Input: part model. Units: mm. Frame: model coordinates. Face numbers are marked on the shaded views. A direction names the side the tool comes from. Give positions to 0.01 mm unless a question says otherwise; leave off trailing zeros. Write each loop counter-clockwise with the first axis right and the second up, starting at its lowest first coordinate (ties: lowest second). Pieces come first, ordered by that corner, then holes. Notation, with made-up numbers: (33.5, 71.5) -> (77.5, 71.5) arc R31 cw to (77.5, 100.5) -> close; hole circle Ø7 at (48, -38). An arc over 180 degrees is marked (long way). Return JSON: item names as keys, results as strings. Group by question number.
Item 1: Section B-B, the plane x = 0. Return loops of the section in (y, z).
Item 2: Line query: line 1 (Y direction, x = -1.1, z = -1.85); line 2 (X direction, y = 2, z = 1.15); line 3 (X direction, y = 2.25, z = 0.55). Output: solid intervals per line, ascending. Write a range as [from, to].
Item 3: Section C-C, the plane y = -0.25. Return loops of the section in (x, z).
Item 4: Mould query, pull axis X, two halves, no side actions, for the marked faces 4, 5 and 6. Classes: released by +X, released by -X, zero draft, split by the parting line, or undercut.
Item 5: Set-up query: the marked faces 1, 2 and 3. Return all of +Z, -Z, +X, -X, +Y, -Y with unobstructed straight access to the full face (end or side cutting, diameter ignored); none if empty.
Item 6: Section A-A, the plane y = 2. Return loops of the section in (x, z).
from build123d import *

# Parameters (mm, degrees)
SKETCH_1_R          = 2.75
EXTRUDE_1_DEPTH     = 3
CUT_EXTRUDE_1_DEPTH = 1.3
FILLET_1_R          = 0.15
SKETCH_5_R          = 1.5
EXTRUDE_2_DEPTH     = 8
CHAMFER_2_SIZE      = 0.28


with BuildPart() as part:
    # 草图1 → 凸台-拉伸1 (new body)
    with BuildSketch(Plane(origin=(0, 0, 0), x_dir=(1, 0, 0), z_dir=(0, 1, 0))):
        with Locations(Location((0, 0, 0), (0, 0, 270))):
            Circle(SKETCH_1_R)
    extrude(amount=EXTRUDE_1_DEPTH)

    # 草图2 → 切除-拉伸1 (cut)
    with BuildSketch(Plane(origin=(0, 3, 0), x_dir=(1, 0, 0), z_dir=(0, 1, 0))):
        Polygon((1.478016689, 0), (0.739008345, 1.28), (-0.739008345, 1.28), (-1.478016689, 0), (-0.739008345, -1.28), (0.739008345, -1.28), align=None)
    extrude(amount=-CUT_EXTRUDE_1_DEPTH, mode=Mode.SUBTRACT)

    # 圆角1
    fillet_1_edges = [part.edges().sort_by_distance(p)[0] for p in [
        (0, 3, -2.75),
    ]]
    fillet(fillet_1_edges, radius=FILLET_1_R)

    # 草图5 → 凸台-拉伸2 (add)
    with BuildSketch(Plane.XZ):
        with Locations(Location((0, 0, 0), (0, 0, 90))):
            Circle(SKETCH_5_R)
    extrude(amount=EXTRUDE_2_DEPTH)

    # 倒角2
    chamfer_2_edges = [part.edges().sort_by_distance(p)[0] for p in [
        (0, -8, -1.5),
    ]]
    chamfer(chamfer_2_edges, length=CHAMFER_2_SIZE)


solid = part.part
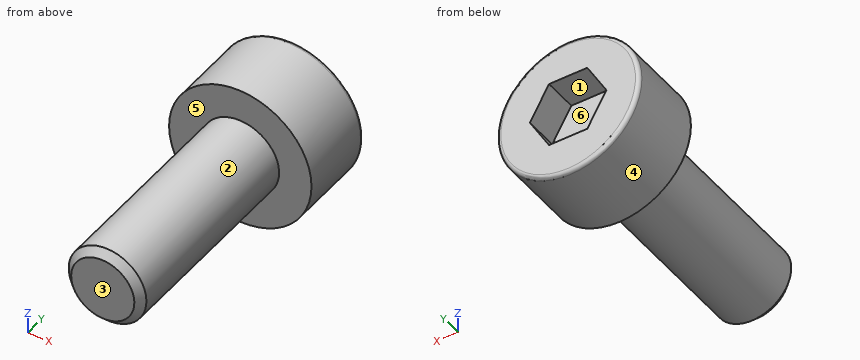
Answer below:
{
 "1": {"outline": "(-8, -1.22) -> (-7.72, -1.5) -> (0, -1.5) -> (0, -2.75) -> (2.85, -2.75) arc R0.15 ccw to (3, -2.6) -> (3, -1.28) -> (1.7, -1.28) -> (1.7, 1.28) -> (3, 1.28) -> (3, 2.6) arc R0.15 ccw to (2.85, 2.75) -> (0, 2.75) -> (0, 1.5) -> (-7.72, 1.5) -> (-8, 1.22) -> close"},
 "2": {"line 1": "y = [0, 3]", "line 2": "x = [-2.5, -0.81], [0.81, 2.5]", "line 3": "x = [-2.69, -1.16], [1.16, 2.69]"},
 "3": {"outline": "circle Ø3 at (0, 0)"},
 "4": {"face 4": "split by the parting line", "face 5": "zero draft", "face 6": "undercut"},
 "5": {"face 1": "+Y", "face 2": "-Y", "face 3": "+Z, -Z, +X, -X, -Y"},
 "6": {"outline": "circle Ø5.5 at (0, 0); hole (-1.48, 0) -> (-0.74, -1.28) -> (0.74, -1.28) -> (1.48, 0) -> (0.74, 1.28) -> (-0.74, 1.28) -> close"}
}
